Build history of the part. All positions in model axes, mm. Face numbers are marked on the shaded views. Round coordinates to 2 decimals unless told otherwise and drop trailing zeros. Write each loop counter-clockwise with the first axis right and the second up, starting at its lowest first coordinate (ties: lowest second). Pieces come first, ordered by that corner, then holes.
Item 1: Band-saw the part on C-C, the plane y = 6. Write the cut outline in (x, z).
Item 2: Band-saw the part on B-B, the plane x = 0. Write the cut outline in (y, z).
Item 3: Band-saw the part on A-A, the plane y = 0. Write the cut outline in (x, z).
Item 4: Band-saw the part on D-D, the plane z = 6.75. Write the cut outline in (x, y), then the cut area to 3 significant figures.
Item 5: Wall check: probe 1 along Z at (x, y) = (26, -0.5); probe 2 along X at (y, z) = (-2, 5.5); probe 3 along Y at (x, z) = (21, 2.5). Give the ranges that are in metal, low to high.
Item 6: Drop flat-ended pins along their axis: pin 1 Ø5 at (x, z) = (32, 3) entering from +Y; pin 2 Ø3 at (y, z) = (4.5, 6) entering from +X; pin 3 Ø3 at (x, z) = (57.5, 8) entering from -Y; pin 4 Ø7 at (x, y) = (69, 2) entering from +Z. Give the stop position or say it passes through.
Item 7: Mould opens along X. For the marked faces 1 and 2 say: +X half, -X half, draft (parallel to the pull), parting line (faces both ways), or undercut.
```python
from build123d import *

# Parameters (mm, degrees)
BASE_EXTRUDE_DEPTH  = 5
SKETCH2_R           = 5
BOSS_EXTRUDE1_DEPTH = 5


with BuildPart() as part:
    # Sketch1 → Base-Extrude (new body)
    with BuildSketch(Plane.XY):
        with BuildLine():
            Line((4.898979486, -5), (85.101020514, -5))
            ThreePointArc((85.101020514, -5), (97, 0), (85.101020514, 5))
            Line((85.101020514, 5), (4.898979486, 5))
            ThreePointArc((4.898979486, 5), (-7, 0), (4.898979486, -5))
        make_face()
    extrude(amount=BASE_EXTRUDE_DEPTH)

    # Sketch2 → Boss-Extrude1 (add)
    with BuildSketch(Plane.XY.offset(5)):
        Circle(SKETCH2_R)
        with Locations((90, 0)):
            Circle(SKETCH2_R)
    extrude(amount=BOSS_EXTRUDE1_DEPTH)


solid = part.part
```
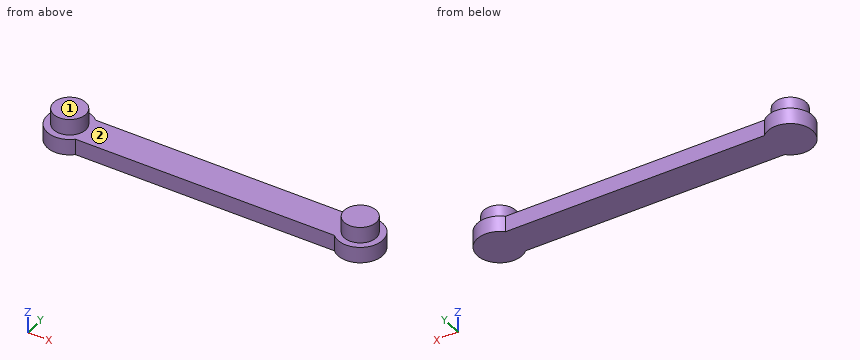
Results:
1. outline: (-3.61, 0) - (3.61, 0) - (3.61, 5) - (-3.61, 5) - close; (86.39, 0) - (93.61, 0) - (93.61, 5) - (86.39, 5) - close
2. outline: (-7, 0) - (7, 0) - (7, 5) - (5, 5) - (5, 10) - (-5, 10) - (-5, 5) - (-7, 5) - close
3. outline: (-7, 0) - (97, 0) - (97, 5) - (95, 5) - (95, 10) - (85, 10) - (85, 5) - (5, 5) - (5, 10) - (-5, 10) - (-5, 5) - (-7, 5) - close
4. outline: circle Ø10 at (0, 0); circle Ø10 at (90, 0)
4. area: 157 mm2
5. probe 1: z = 0 to 5
5. probe 2: x = -4.58 to 4.58, 85.42 to 94.58
5. probe 3: y = -5 to 5
6. pin 1: stops at y = 5
6. pin 2: stops at x = 96.13
6. pin 3: passes through
6. pin 4: stops at z = 5
7. face 1: draft
7. face 2: undercut
